from build123d import *

# Parameters (mm, degrees)
SKETCH2_R     = 10
CHAMFER1_SIZE = 5


with BuildPart() as part:
    # Sweep1: sweep along a path in Sketch4
    with BuildLine(Plane(origin=(0, 0, 0), x_dir=(0, 0, -1), z_dir=(1, 0, 0))) as sweep1_path:
        Line((0, 0), (-34, 0))
        ThreePointArc((-34, 0), (-44.606601718, 4.393398282), (-49, 15))
        Line((-49, 15), (-49, 111))
        ThreePointArc((-49, 111), (-44.606601718, 121.606601718), (-34, 126))
        Line((-34, 126), (36, 126))
        ThreePointArc((36, 126), (46.606601718, 121.606601718), (51, 111))
        Line((51, 111), (51, 15))
        ThreePointArc((51, 15), (46.606601718, 4.393398282), (36, 0))
        Line((36, 0), (2, 0))
    # Sketch2 → Sweep1 (sweep)
    with BuildSketch(Plane.XY):
        Circle(SKETCH2_R)
    sweep(path=sweep1_path.line)

    # Chamfer1
    chamfer1_edges = [part.edges().sort_by_distance(p)[0] for p in [
        (-10, 0, -2),
        (-10, 0, 0),
    ]]
    chamfer(chamfer1_edges, length=CHAMFER1_SIZE)


solid = part.part
Build history of the part. All positions in model axes, mm. A direction names the side the tool comes from. Coordinates: 2 decimals unless noted, no trailing zeros. Write each loop counter-clockwise with the first axis right and the second up, starting at its lowest first coordinate (ties: lowest second). Pieces come first, ordered by that corner, then holes. Notation, with made-up numbers: (-35.5, -20) -> (20.5, -20) arc R29 cw to (20.5, 4) -> close; hole circle Ø4 at (58, 40.25). An arc over 180 degrees is marked (long way). Use CSV: the item, a comma, the result in double quotes. Start each with the question number.
Q1. Drill centre lines: probe 1 along Y at (x, z) = (-0.5, -31.5); probe 2 along Y at (x, z) = (-7.25, 30); probe 3 along Z at (x, y) = (-5.25, 91.5). Where is each one in solid material? Low to high.
Q2. Cut at A-A, the plane z = 31. List the corners of the cut face in (x, y).
Q3. Cut at C-C, the plane y = 61.5. List the corners of the cut face in (x, z), then the cut area to 3 significant figures.
Q4. 3-axis set-ups, long thin cutter, end or side, ignore diameter. For faces 1 (the flat face through (0, 0, 0)), 2 (the cylindrical face through (-2.17, 63.67, 58.76)): which of +Z, -Z, +X, -X, +Y, -Y reach the whole face in a straight line?
Q5. Flat gauge pins, fed straight in: pin 1 Ø8 at (x, y) = (1, 0) entering from -Z; pin 2 Ø5 at (x, z) = (-1.5, -46) entering from -Y; pin 3 Ø5 at (y, z) = (8, 18.5) entering from +X. Where does each tip first touch, or does it go through?
Q6. Cut at B-B, the plane x = 0. List the corners of the cut face in (y, z).
Checked values:
1,probe 1,"y = -9.99 to 9.99, 116.01 to 135.99"
1,probe 2,"y = -6.89 to 6.89, 119.11 to 132.89"
1,probe 3,"z = -59.51 to -42.49, 40.49 to 57.51"
2,outline,"circle Ø20 at (0, 0); circle Ø20 at (0, 126)"
3,outline,"circle Ø20 at (0, -51); circle Ø20 at (0, 49)"
3,area,"628 mm²"
4,face 1,"+X, -X, -Y"
4,face 2,"none"
5,pin 1,"stops at z = -58.42"
5,pin 2,"stops at y = -8.78"
5,pin 3,"stops at x = 8.35"
6,outline,"(-10, -36) arc R25 ccw to (15, -61) -> (111, -61) arc R25 ccw to (136, -36) -> (136, 34) arc R25 ccw to (111, 59) -> (15, 59) arc R25 ccw to (-10, 34) -> (-10, 5) -> (-5, 0) -> (5, 0) -> (10, 5) -> (10, 34) arc R5 cw to (15, 39) -> (111, 39) arc R5 cw to (116, 34) -> (116, -36) arc R5 cw to (111, -41) -> (15, -41) arc R5 cw to (10, -36) -> (10, -7) -> (5, -2) -> (-5, -2) -> (-10, -7) -> close"
